Geometry: final body of the model. Coordinates: model frame, mm. Give positions to 0.01 mm unless a question says otherwise; leave off trailing zeros. Write each loop counter-clockwise with the first axis right and the second up, starting at its lowest first coordinate (ties: lowest second). Pieces come first, ordered by that corner, then holes.
Q1. Section A-A (x = 45). Return the cut outline in (y, z), plus the area to 3 significant figures.
Q2. Section B-B (y = 0). Return the cut outline in (x, z).
Q3. Section C-C (z = 1.45). Return the cut outline in (x, y), plus the area to 3 significant figures.
Q4. Line query: line 1 (X direction, y = 2.5, z = 1.9); line 2 (Y direction, x = -45, z = 0.9); line 3 (X direction, y = -10.25, z = 0.7). Output: solid intervals per line, ascending.
Q5. Mould query, pull axis Y, two halves, no side actions, for faces 1 (the cylindrical face through (-39.505, 0.242, 0.986)), 2 (the cylindrical face through (-59, -13, 1)), 3 (the flat face through (-1, 15, 1)). Classes: +Y half, -Y half, draft (parallel to the pull), parting line (faces both ways), or undercut.
from build123d import *

# Parameters (mm, degrees)
SKETCH_1_W          = 120
SKETCH_1_H          = 30
EXTRUDE_1_DEPTH     = 2
SKETCH_2_R          = 5.5
CUT_EXTRUDE_1_DEPTH = 10
FILLET_1_R          = 5


with BuildPart() as part:
    # 草图1 → 凸台-拉伸1 (new body)
    with BuildSketch(Plane.XY):
        Rectangle(SKETCH_1_W, SKETCH_1_H)
    extrude(amount=EXTRUDE_1_DEPTH)

    # 草图2 → 切除-拉伸1 (cut)
    with BuildSketch(Plane(origin=(0, 0, 0), x_dir=(-1, 0, 0), z_dir=(0, 0, -1))):
        with Locations((45, 0)):
            Circle(SKETCH_2_R)
        with Locations((-45, 0)):
            Circle(SKETCH_2_R)
    extrude(amount=-CUT_EXTRUDE_1_DEPTH, mode=Mode.SUBTRACT)

    # 圆角1
    fillet_1_edges = [part.edges().sort_by_distance(p)[0] for p in [
        (60, -15, 1),
        (-60, -15, 1),
        (-60, 15, 1),
        (60, 15, 1),
    ]]
    fillet(fillet_1_edges, radius=FILLET_1_R)


solid = part.part
Computed:
1. outline: (-15, 0) - (-5.5, 0) - (-5.5, 2) - (-15, 2) - close; (5.5, 0) - (15, 0) - (15, 2) - (5.5, 2) - close
1. area: 38.0 mm2
2. outline: (-60, 0) - (-50.5, 0) - (-50.5, 2) - (-60, 2) - close; (-39.5, 0) - (39.5, 0) - (39.5, 2) - (-39.5, 2) - close; (50.5, 0) - (60, 0) - (60, 2) - (50.5, 2) - close
3. outline: (-60, -10) arc R5 ccw to (-55, -15) - (55, -15) arc R5 ccw to (60, -10) - (60, 10) arc R5 ccw to (55, 15) - (-55, 15) arc R5 ccw to (-60, 10) - close; hole circle Ø11 at (-45, 0); hole circle Ø11 at (45, 0)
3. area: 3,390 mm2
4. line 1: x = -60 to -49.9, -40.1 to 40.1, 49.9 to 60
4. line 2: y = -15 to -5.5, 5.5 to 15
4. line 3: x = -59.99 to 59.99
5. face 1: undercut
5. face 2: -Y half
5. face 3: +Y half
